Check sheet for the modelled part. Datum: model origin and axes. Units: mm. A direction names the side the tool comes from. Round coordinates to 2 decimals unless told otherwise and drop trailing zeros. Loops run counter-clockwise (first coordinate to the right, second up) from the corner with the lowest first, then second, coordinate; pieces in that order, holes last. Notation, with made-up numbers: M 37,-32 L 62,-32 A13 ccw 62,-23 Z; hole C -23,78.5 d5. An arc over 180 degrees is marked long. One line per question, with ' | ' between items. Start each with the question number.
(1) Section check C-C (x = -33). Record the boundary of the cut face in (y, z), and give its area (3 significant figures).
(2) Thickness scan on probe 1 along Z at (x, y) = (-17.5, -1.9); probe 2 along X at (y, z) = (-3.1, -17.5); probe 3 along Z at (x, y) = (-34, 24). Record the ranges inside material, lowest first. Write a range as [from, to].
(3) Section check A-A (x = 22.5). Record the boundary of the cut face in (y, z).
(4) Go/stop test with flat-tipped pins: P1, Ø8, axis at x = 3, z = -16.5, coming from the +Y side; P2, Ø10.5, axis at y = 20, z = -7.5, coming from the +X side; P3, Ø6, axis at x = -13.5, z = -16.5, coming from the +Y side. Record where each tip stops, or that it passes through.
(5) Tool access check on faces 1 (the face through (-27.5, 22, 0)), 2 (the face through (-32, 18, 20)), 3 (the face through (-32.6, 39, 31.5)). Record the directions out of +Z, -Z, +X, -X, +Y, -Y that give a thin tool (end or side, any length) a straight path to the whole face; none if there is none.
(6) Section check B-B (y = 24.5). Record the boundary of the cut face in (x, z).
(7) Section check D-D (z = -5). Record the boundary of the cut face in (x, y).
(8) Draft check along X on faces 4 (the face through (-15, 4, -32.5)), 5 (the face through (25.82, -2.27, 14.46)), 6 (the face through (37, 0, -31)), 7 (the face through (-37.5, 17, 0)). Enter one of: +X half, -X half, draft (parallel to the pull), parting line (faces both ways), or undercut.
```python
from build123d import *

# Parameters (mm, degrees)
SKETCH_2_W                   = 75
SKETCH_2_H                   = 65
EXTRUDE_1_DEPTH              = 5
SKETCH_3_W                   = 10
SKETCH_3_H                   = 65
EXTRUDE_2_DEPTH              = 45
HOLE_WIZARD_M8_1_D           = 9
HOLE_WIZARD_M8_1_CSINK_D     = 17.92
HOLE_WIZARD_M8_1_CSINK_ANGLE = 90
CUT_EXTRUDE_1_DEPTH          = 45
CHAMFER_1_SIZE               = 2


with BuildPart() as part:
    # 草图2 → 凸台-拉伸1 (new, symmetric)
    with BuildSketch(Plane(origin=(0, 0, 0), x_dir=(1, 0, 0), z_dir=(0, 1, 0))):
        Rectangle(SKETCH_2_W, SKETCH_2_H)
    extrude(amount=EXTRUDE_1_DEPTH, both=True)

    # 草图3 → 凸台-拉伸2 (add)
    with BuildSketch(Plane.XZ.offset(5)):
        with Locations((-32.5, 0)):
            Rectangle(SKETCH_3_W, SKETCH_3_H)
    extrude(amount=-EXTRUDE_2_DEPTH)

    # M8 六角凹锥坑螺钉的锥形沉头孔1 (through all)
    with Locations(Plane(origin=(0, 5, 0), x_dir=(1, 0, 0), z_dir=(0, 1, 0))):
        with Locations((22.5, 17.5), (-17.5, 17.5), (-17.5, -17.5), (22.5, -17.5)):
            CounterSinkHole(HOLE_WIZARD_M8_1_D / 2, HOLE_WIZARD_M8_1_CSINK_D / 2, counter_sink_angle=HOLE_WIZARD_M8_1_CSINK_ANGLE)

    # 草图6 → 切除-拉伸1 (cut)
    with BuildSketch(Plane(origin=(-27.5, 0, 0), x_dir=(0, 0, -1), z_dir=(1, 0, 0))):
        with BuildLine():
            Line((24.5, 27.5), (24.5, 22.5))
            ThreePointArc((24.5, 22.5), (20, 18), (15.5, 22.5))
            Line((15.5, 22.5), (15.5, 27.5))
            ThreePointArc((15.5, 27.5), (20, 32), (24.5, 27.5))
        make_face()
        with BuildLine():
            Line((-24.5, 27.5), (-24.5, 22.5))
            ThreePointArc((-24.5, 22.5), (-20, 18), (-15.5, 22.5))
            Line((-15.5, 22.5), (-15.5, 27.5))
            ThreePointArc((-15.5, 27.5), (-20, 32), (-24.5, 27.5))
        make_face()
    extrude(amount=-CUT_EXTRUDE_1_DEPTH, mode=Mode.SUBTRACT)

    # 倒角1
    chamfer_1_edges = [part.edges().sort_by_distance(p)[0] for p in [
        (-32.5, 40, -32.5),
        (-32.5, 40, 32.5),
        (37.5, 0, 32.5),
        (37.5, 0, -32.5),
    ]]
    chamfer(chamfer_1_edges, length=CHAMFER_1_SIZE)


solid = part.part
```
The answers:
1) outline: M -5,-32.5 L 38,-32.5 L 40,-30.5 L 40,30.5 L 38,32.5 L -5,32.5 Z; hole M 22.5,-24.5 L 27.5,-24.5 A4.5 ccw 27.5,-15.5 L 22.5,-15.5 A4.5 ccw Z; hole M 22.5,15.5 L 27.5,15.5 A4.5 ccw 27.5,24.5 L 22.5,24.5 A4.5 ccw Z | area: 2,700 mm²
2) probe 1: [-32.5, -22], [-13, 13], [22, 32.5] | probe 2: [-37.5, -22], [-13, 18], [27, 37.5] | probe 3: [-32.5, -24.5], [-15.5, 15.5], [24.5, 32.5]
3) outline: M -5,-32.5 L 5,-32.5 L 5,-26.46 L 0.54,-22 L -5,-22 Z; M -5,-13 L 0.54,-13 L 5,-8.54 L 5,8.54 L 0.54,13 L -5,13 Z; M -5,22 L 0.54,22 L 5,26.46 L 5,32.5 L -5,32.5 Z
4) P1: y = 5 | P2: x = -27.5 | P3: y = 3.16
5) face 1: +Z, -Z, +X, +Y | face 2: +X, -X | face 3: +Z, +X, -X, +Y
6) outline: M -37.5,-32.5 L -27.5,-32.5 L -27.5,-24.5 L -37.5,-24.5 Z; M -37.5,-15.5 L -27.5,-15.5 L -27.5,15.5 L -37.5,15.5 Z; M -37.5,24.5 L -27.5,24.5 L -27.5,32.5 L -37.5,32.5 Z
7) outline: M -37.5,-5 L 37.5,-5 L 37.5,5 L -27.5,5 L -27.5,40 L -37.5,40 Z
8) face 4: draft | face 5: undercut | face 6: +X half | face 7: -X half
